Check sheet for the modelled part. Datum: model origin and axes. Units: mm. A direction names the side the tool comes from. Round coordinates to 2 decimals unless told otherwise and drop trailing zeros. Loops run counter-clockwise (first coordinate to the right, second up) from the corner with the lowest first, then second, coordinate; pieces in that order, holes last. Notation, with made-up numbers: (58.5, 72.5) - (77.5, 72.5) arc R25 ccw to (77.5, 85.5) - close; hole circle Ø4 at (38, -13.75). An arc over 180 degrees is marked (long way). Put each result on its own line as item: value. Start each with the question number.
Item 1: Section check B-B, the plane z = 22. Record the cut outline in (x, y).
Item 2: Tool access check on faces 1 (the flat face through (0, 20, 27)), 2 (the flat face through (19, 8, 30)), 3 (the cylindrical face through (36.503, 0.154, 4.93)), 4 (the flat face through (-14, -14, 27)), 5 (the flat face through (20, -4, 28)). Record the directions out of +Z, -Z, +X, -X, +Y, -Y that give a thin tool (end or side, any length) a straight path to the whole face; none if there is none.
Item 3: Section check C-C, the plane z = 2.25. Record the cut outline in (x, y).
Item 4: Gauge pin test, flat ends, axial feed: pin 1 Ø1.5 at (x, z) = (21.5, 28.5) entering from -Y; pin 2 Ø4 at (y, z) = (-19, 22.5) entering from +X; pin 3 Ø5.5 at (x, y) = (-14, 16.5) entering from +Z; pin 4 Ø1.5 at (x, z) = (-21.5, 28) entering from +Y. Record the tip position at first contact, or that the pin passes through.
Item 5: Draft check along X on faces 6 (the flat face through (-12, -11, 0)), 7 (the cylindrical face through (-0.46, 43.47, 4.93)). Enter one of: pulls with the +X half, pulls with the -X half, needs draft (parallel to the pull), parting line crosses it, or undercut.
Item 6: Section check D-D, the plane y = 40. Record the cut outline in (x, z), and give its area (3 significant figures).
Item 7: Material ranges on line 1 along Y through (x, z) = (0, 4); line 2 along Y through (x, z) = (0, 13); line 3 along X through (y, z) = (-0.5, 24.5), recorded low to high.
Item 8: Section check A-A, the plane x = 39. Record the cut outline in (y, z).
from build123d import *

# Parameters (mm, degrees)
SKETCH_1_R          = 52.5
SKETCH_1_R_2        = 16
SKETCH_1_R_3        = 3.5
EXTRUDE_1_DEPTH     = 10
SKETCH_2_R          = 24
SKETCH_2_R_2        = 16
EXTRUDE_2_DEPTH     = 20
CUT_EXTRUDE_START   = -3
CUT_EXTRUDE_2_DEPTH = 3


with BuildPart() as part:
    # 草图1 → 凸台-拉伸1 (new body)
    with BuildSketch(Plane.XY):
        Circle(SKETCH_1_R)
        Circle(SKETCH_1_R_2, mode=Mode.SUBTRACT)
        with Locations((0, 40)):
            Circle(SKETCH_1_R_3, mode=Mode.SUBTRACT)
        with Locations((40, 0)):
            Circle(SKETCH_1_R_3, mode=Mode.SUBTRACT)
        with Locations((0, -40)):
            Circle(SKETCH_1_R_3, mode=Mode.SUBTRACT)
        with Locations((-40, 0)):
            Circle(SKETCH_1_R_3, mode=Mode.SUBTRACT)
    extrude(amount=EXTRUDE_1_DEPTH)

    # 草图2 → 凸台-拉伸2 (add)
    with BuildSketch(Plane.XY.offset(10)):
        Circle(SKETCH_2_R)
        Circle(SKETCH_2_R_2, mode=Mode.SUBTRACT)
    extrude(amount=EXTRUDE_2_DEPTH)

    # 草图3 → 切除-拉伸2 (cut)
    with BuildSketch(Plane.XY.offset(30).offset(CUT_EXTRUDE_START)):
        with BuildLine():
            Line((-4, 23.664319132), (-4, 15.491933385))
            ThreePointArc((-4, 15.491933385), (0, 16), (4, 15.491933385))
            Line((4, 15.491933385), (4, 23.664319132))
            ThreePointArc((4, 23.664319132), (0, 24), (-4, 23.664319132))
        make_face()
        with BuildLine():
            Line((13.904773406, 19.561627655), (8.126024025, 13.782878275))
            ThreePointArc((8.126024025, 13.782878275), (11.313708499, 11.313708499), (13.782878275, 8.126024025))
            Line((13.782878275, 8.126024025), (19.561627655, 13.904773406))
            ThreePointArc((19.561627655, 13.904773406), (16.970562748, 16.970562748), (13.904773406, 19.561627655))
        make_face()
        with BuildLine():
            Line((23.664319132, 4), (15.491933385, 4))
            ThreePointArc((15.491933385, 4), (16, 0), (15.491933385, -4))
            Line((15.491933385, -4), (23.664319132, -4))
            ThreePointArc((23.664319132, -4), (24, 0), (23.664319132, 4))
        make_face()
        with BuildLine():
            Line((19.561627655, -13.904773406), (13.782878275, -8.126024025))
            ThreePointArc((13.782878275, -8.126024025), (11.313708499, -11.313708499), (8.126024025, -13.782878275))
            Line((8.126024025, -13.782878275), (13.904773406, -19.561627655))
            ThreePointArc((13.904773406, -19.561627655), (16.970562748, -16.970562748), (19.561627655, -13.904773406))
        make_face()
        with BuildLine():
            Line((4, -23.664319132), (4, -15.491933385))
            ThreePointArc((4, -15.491933385), (0, -16), (-4, -15.491933385))
            Line((-4, -15.491933385), (-4, -23.664319132))
            ThreePointArc((-4, -23.664319132), (0, -24), (4, -23.664319132))
        make_face()
        with BuildLine():
            Line((-13.904773406, -19.561627655), (-8.126024025, -13.782878275))
            ThreePointArc((-8.126024025, -13.782878275), (-11.313708499, -11.313708499), (-13.782878275, -8.126024025))
            Line((-13.782878275, -8.126024025), (-19.561627655, -13.904773406))
            ThreePointArc((-19.561627655, -13.904773406), (-16.970562748, -16.970562748), (-13.904773406, -19.561627655))
        make_face()
        with BuildLine():
            Line((-23.664319132, -4), (-15.491933385, -4))
            ThreePointArc((-15.491933385, -4), (-16, 0), (-15.491933385, 4))
            Line((-15.491933385, 4), (-23.664319132, 4))
            ThreePointArc((-23.664319132, 4), (-24, 0), (-23.664319132, -4))
        make_face()
        with BuildLine():
            Line((-19.561627655, 13.904773406), (-13.782878275, 8.126024025))
            ThreePointArc((-13.782878275, 8.126024025), (-11.313708499, 11.313708499), (-8.126024025, 13.782878275))
            Line((-8.126024025, 13.782878275), (-13.904773406, 19.561627655))
            ThreePointArc((-13.904773406, 19.561627655), (-16.970562748, 16.970562748), (-19.561627655, 13.904773406))
        make_face()
    extrude(amount=CUT_EXTRUDE_2_DEPTH, mode=Mode.SUBTRACT)


solid = part.part
Check result:
1. outline: circle Ø48 at (0, 0); hole circle Ø32 at (0, 0)
2. face 1: +Z, +Y, -Y
2. face 2: +Z, +X, -X, +Y, -Y
2. face 3: +Z, -Z
2. face 4: +Z
2. face 5: +Z, +X, -X
3. outline: circle Ø105 at (0, 0); hole circle Ø7 at (-40, 0); hole circle Ø32 at (0, 0); hole circle Ø7 at (0, -40); hole circle Ø7 at (0, 40); hole circle Ø7 at (40, 0)
4. pin 1: y = -12.06
4. pin 2: x = 16.94
4. pin 3: z = 30
4. pin 4: y = 12.06
5. face 6: needs draft
5. face 7: undercut
6. outline: (-34, 0) - (-3.5, 0) - (-3.5, 10) - (-34, 10) - close; (3.5, 0) - (34, 0) - (34, 10) - (3.5, 10) - close
6. area: 610 mm²
7. line 1: -52.5 to -43.5, -36.5 to -16, 16 to 36.5, 43.5 to 52.5
7. line 2: -24 to -16, 16 to 24
7. line 3: -23.99 to -15.99, 15.99 to 23.99
8. outline: (-35.15, 0) - (-3.35, 0) - (-3.35, 10) - (-35.15, 10) - close; (3.35, 0) - (35.15, 0) - (35.15, 10) - (3.35, 10) - close
